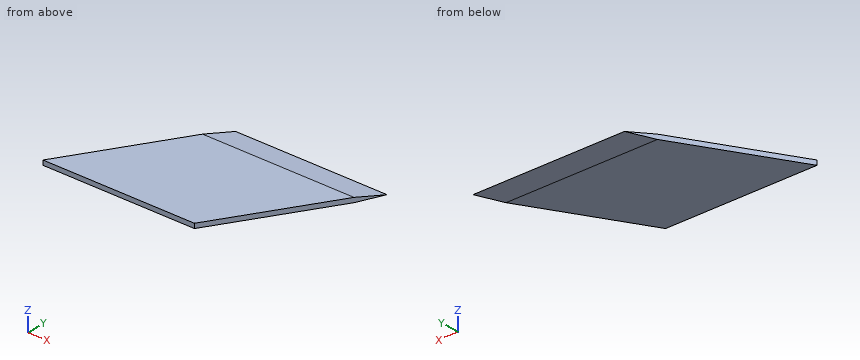
from build123d import *

# Parameters (mm, degrees)
BOSS_EXTRUDE1_DEPTH = 0.6
CUT_EXTRUDE1_DEPTH  = 35.825831243


with BuildPart() as part:
    # Sketch1 → Boss-Extrude1 (new body)
    with BuildSketch(Plane.XY):
        Polygon((0, 0), (10.103629711, 17.5), (30.103629711, 17.5), (20, 0), align=None)
    extrude(amount=BOSS_EXTRUDE1_DEPTH)

    # Sketch2 → Cut-Extrude1 (cut, through all)
    with BuildSketch(Plane(origin=(0, 0, 0), x_dir=(0, 0, -1), z_dir=(1, 0, 0))):
        Polygon((-0.3, 17.5), (0, 14.5), (0, 17.5), align=None)
    cut_extrude1 = extrude(amount=CUT_EXTRUDE1_DEPTH, mode=Mode.SUBTRACT)

    # Mirror1: Cut-Extrude1 across plane
    add(cut_extrude1.mirror(Plane(origin=(0, 0, 0.3), x_dir=(1, 0, 0), z_dir=(0, 0, -1))), mode=Mode.SUBTRACT)


solid = part.part
Work out the finished part from the listing and answer in its coordinate system (mm). Round coordinates to 2 decimals unless told otherwise and drop trailing zeros. Order: outer loops, then holes, each group sorted by start corner. A loop starts at its lowest first (then second) coordinate and runs counter-clockwise, first axis right, second up. Notation, with made-up numbers: M -37.75,-34.75 L 21.25,-34.75 A9 ccw 21.25,-25.75 Z; hole C 48,-18.5 d10. An arc over 180 degrees is marked long. Put each result on its own line as item: value. Start each with the question number.
Q1. A flat-ended cylindrical pin translates along its axis: pin 1 (1.5 mm diameter, centred on x = 22.5, y = 15.5, fed in from +Z) (3 decimals). Find the tip coordinate at first contact, or state that the pin passes through.
Q2. Section C-C, the plane z = 0.1 is taken. Write down the section's boundary in (x, y), and give its area (3 significant figures).
Q3. Straight lines are drawn through the part: L1, parallel to X at y = 13.25, z = 0.2; L2, parallel to X at y = 11, z = 0.2; L3, parallel to Y at x = 6, z = 0.1. For each, find the intervals that lie inside material, in ascending order. Write a range as [from, to].
Q4. Section D-D, the plane x = 26 is taken. Write down the section's boundary in (y, z), and give its area (3 significant figures).
Q5. Section B-B, the plane y = 3 is taken. Write down the section's boundary in (x, z).
Q6. Section A-A, the plane x = 17 is taken. Write down the section's boundary in (y, z).
Findings below:
1. pin 1: stops at z = 0.575
2. outline: M 0,0 L 20,0 L 28.95,15.5 L 8.95,15.5 Z
2. area: 310 mm^2
3. L1: x = [7.65, 27.65]
3. L2: x = [6.35, 26.35]
3. L3: y = [0, 10.39]
4. outline: M 10.39,0 L 14.5,0 L 17.5,0.3 L 14.5,0.6 L 10.39,0.6 Z
4. area: 3.36 mm^2
5. outline: M 1.73,0 L 21.73,0 L 21.73,0.6 L 1.73,0.6 Z
6. outline: M 0,0 L 14.5,0 L 17.5,0.3 L 14.5,0.6 L 0,0.6 Z
